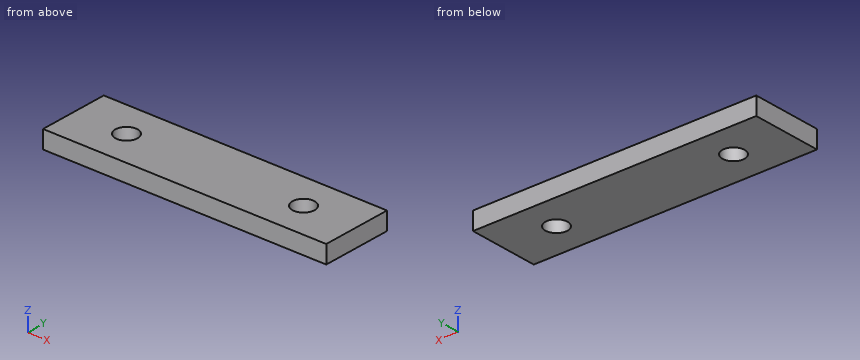
```python
from build123d import *

# Parameters (mm, degrees)
SKETCH1_W                    = 160
SKETCH1_H                    = 40
BOSS_EXTRUDE1_DEPTH          = 5
F_12_5_12_5_DIAMETER_HOLE1_D = 12.5


with BuildPart() as part:
    # Sketch1 → Boss-Extrude1 (new, symmetric)
    with BuildSketch(Plane.XY):
        Rectangle(SKETCH1_W, SKETCH1_H)
    extrude(amount=BOSS_EXTRUDE1_DEPTH, both=True)

    # Ø12.5 (12.5) Diameter Hole1 (through all)
    with Locations(Plane.XY.offset(5)):
        with Locations((-50, 0), (50, 0)):
            Hole(F_12_5_12_5_DIAMETER_HOLE1_D / 2)


solid = part.part
```
Work out the finished part from the listing and answer in its coordinate system (mm). Round coordinates to 2 decimals unless told otherwise and drop trailing zeros. Write each loop counter-clockwise with the first axis right and the second up, starting at its lowest first coordinate (ties: lowest second). Pieces come first, ordered by that corner, then holes. Notation, with made-up numbers: (52, 54.5) - (87, 54.5) arc R21 cw to (87, 64.5) - close; hole circle Ø9 at (82.5, -29.5). An arc over 180 degrees is marked (long way). Return JSON: item names as keys, results as strings. Group by question number.
Q1. The part is cut by section A-A on y = 0. Write down the section's boundary in (x, z).
Q2. This flat-tipped pin is pushed along its axis until it touches: pin 1 Ø10 at (x, y) = (50, 0) entering from -Z. Where does it stop, or does it pass through?
Q3. The part is cut by section B-B on x = 50. Write down the section's boundary in (y, z), then the cut area to 3 significant figures.
Q4. The part is cut by section C-C on z = -2. Write down the section's boundary in (x, y).
Q5. Find the intervals of material crossed by L1, parallel to Y at x = 50, z = 2.25; L2, parallel to X at y = 2, z = -3; L3, parallel to X at y = 1, z = 3.25, in increasing order.
Solved:
{
 "1": {"outline": "(-80, -5) - (-56.25, -5) - (-56.25, 5) - (-80, 5) - close; (-43.75, -5) - (43.75, -5) - (43.75, 5) - (-43.75, 5) - close; (56.25, -5) - (80, -5) - (80, 5) - (56.25, 5) - close"},
 "2": {"pin 1": "through"},
 "3": {"outline": "(-20, -5) - (-6.25, -5) - (-6.25, 5) - (-20, 5) - close; (6.25, -5) - (20, -5) - (20, 5) - (6.25, 5) - close", "area": "275 mm²"},
 "4": {"outline": "(-80, -20) - (80, -20) - (80, 20) - (-80, 20) - close; hole circle Ø12.5 at (-50, 0); hole circle Ø12.5 at (50, 0)"},
 "5": {"L1": "-20 to -6.25, 6.25 to 20", "L2": "-80 to -55.92, -44.08 to 44.08, 55.92 to 80", "L3": "-80 to -56.17, -43.83 to 43.83, 56.17 to 80"}
}
